Can you work these out from the model? Positions are in its coordinate system, mm. A direction names the side the tool comes from. Coordinates: 2 decimals unless noted, no trailing zeros. Order: outer loops, then holes, each group sorted by start corner. A loop starts at its lowest first (then second) coordinate and runs counter-clockwise, first axis right, second up. Notation, with made-up numbers: (56, -6) -> (89, -6) arc R17 cw to (89, 4) -> close; hole circle Ø1 at (-14.75, 35.25). An arc over 180 degrees is marked (long way). Use a Markdown table: item, result. Add a question column.
1. Suppose I cut it at A-A, the plane z = 112. List the corners of the cut face in (x, y) for me.
2. For faces 1 (the flat face through (30, 0, 3)), 2 (the flat face through (26, 0, 3)), which set-ups out of +Z, -Z, +X, -X, +Y, -Y let a thin tool reach every point of the face, with its end or its side?
3. We'd pull the mould along Y, two halves only. Please class faces 3 (the flat face through (-27, 0, -240)), 4 (the flat face through (0, 26, 3)), 5 (the flat face through (0, 30, 3)): pulls with the +Y half, pulls with the -Y half, needs draft (parallel to the pull), parting line crosses it, or undercut.
4. If I drill on line 1 along X through (y, z) = (-3.5, 142.5); line 2 along Y through (x, z) = (-25, 33), over which ranges is the centre line in solid material (lowest first)? Write a range as from..to.
5. Suppose I cut it at B-B, the plane y = 3. List the corners of the cut face in (x, z) for me.
6. For pin 1 Ø12 at (x, y) = (20.5, -18) entering from -Z; pin 2 Ø5 at (x, y) = (-22.5, -6.5) entering from -Z, each with a flat end and sliding along its axis, tell me the tip position at first contact or that it passes through.
```python
from build123d import *

# Parameters (mm, degrees)
SKETCH1_W           = 60
SKETCH1_H           = 60
SKETCH1_W_2         = 52
SKETCH1_H_2         = 52
BOSS_EXTRUDE1_DEPTH = 240
FILLET1_R           = 6
FILLET2_R           = 3


with BuildPart() as part:
    # Sketch1 → Boss-Extrude1 (new, symmetric)
    with BuildSketch(Plane.XY):
        Rectangle(SKETCH1_W, SKETCH1_H)
        Rectangle(SKETCH1_W_2, SKETCH1_H_2, mode=Mode.SUBTRACT)
    extrude(amount=BOSS_EXTRUDE1_DEPTH, both=True)

    # Fillet1
    fillet1_edges = [part.edges().sort_by_distance(p)[0] for p in [
        (30, -30, 0),
        (-30, -30, 0),
        (-30, 30, 0),
        (30, 30, 0),
    ]]
    fillet(fillet1_edges, radius=FILLET1_R)

    # Fillet2
    fillet2_edges = [part.edges().sort_by_distance(p)[0] for p in [
        (26, -26, 0),
        (26, 26, 0),
        (-26, 26, 0),
        (-26, -26, 0),
    ]]
    fillet(fillet2_edges, radius=FILLET2_R)


solid = part.part
```
Worked out:
| question | item | result |
|---|---|---|
| 1 | outline | (-30, -24) arc R6 ccw to (-24, -30) -> (24, -30) arc R6 ccw to (30, -24) -> (30, 24) arc R6 ccw to (24, 30) -> (-24, 30) arc R6 ccw to (-30, 24) -> close; hole (-26, -23) arc R3 ccw to (-23, -26) -> (23, -26) arc R3 ccw to (26, -23) -> (26, 23) arc R3 ccw to (23, 26) -> (-23, 26) arc R3 ccw to (-26, 23) -> close |
| 2 | face 1 | +Z, -Z, +X, +Y, -Y |
| 2 | face 2 | +Z, -Z |
| 3 | face 3 | needs draft |
| 3 | face 4 | undercut |
| 3 | face 5 | pulls with the +Y half |
| 4 | line 1 | x = -30..-26, 26..30 |
| 4 | line 2 | y = -29.92..-25.24, 25.24..29.92 |
| 5 | outline | (-30, -240) -> (-26, -240) -> (-26, 240) -> (-30, 240) -> close; (26, -240) -> (30, -240) -> (30, 240) -> (26, 240) -> close |
| 6 | pin 1 | stops at z = -240 |
| 6 | pin 2 | passes through |
